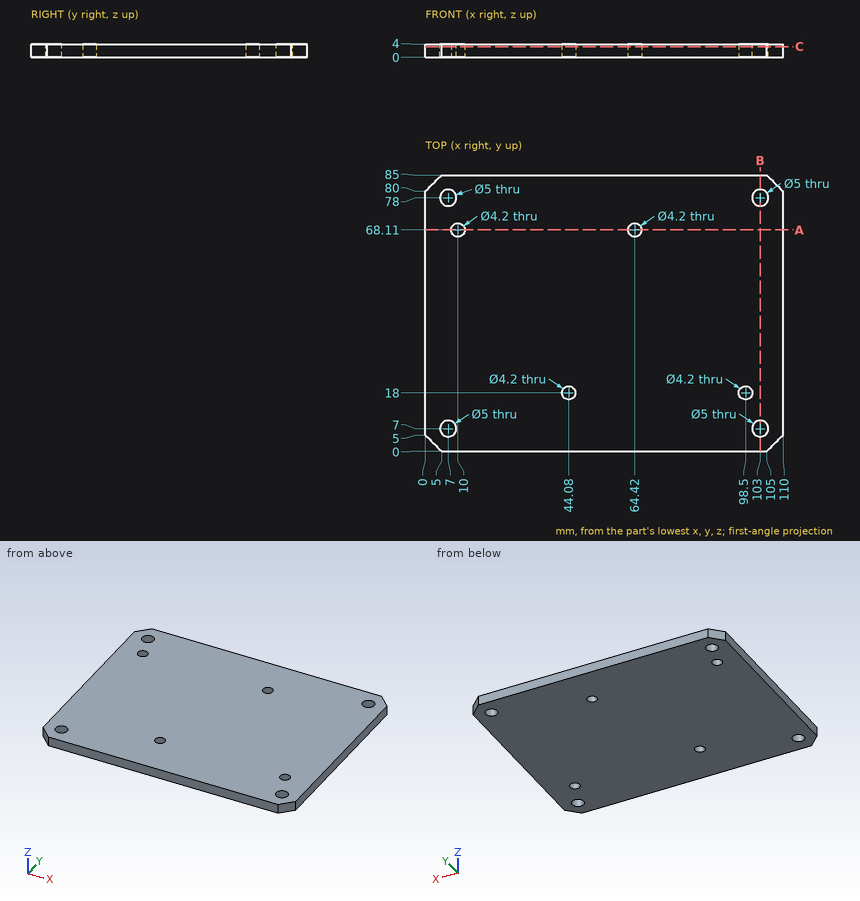
Could you check a few things on this drawing? It's one solid part, dimensions in mm from its lowest x, y, z. Give positions to 0.01 mm unless a question says otherwise; leave off trailing zeros. Write each loop counter-clockwise with the first axis right and the second up, starting at its lowest first coordinate (ties: lowest second). Pieces come first, ordered by that corner, then holes. Notation, with made-up numbers: (1.25, -29.5) - (27.25, -29.5) arc R22 cw to (27.25, -13.5) - close; hole circle Ø3 at (18.5, -28.5). An arc over 180 degrees is marked (long way). Use CSV: the item, a comma, the result in double quotes. Start each with the question number.
Item 1: If I drill on line 1 along Y through (x, z) = (7, 1.8); line 2 along Y through (x, z) = (98.5, 1.3); line 3 along Y through (x, z) = (64.42, 1.8), over which ranges is the centre line in solid material (lowest first)?
Item 2: I want a section at A-A, the plane y = 68.11. Please give me the cut outline in (x, z), then the cut area to 3 significant figures.
Item 3: I want a section at B-B, the plane x = 103. Please give me the cut outline in (y, z), then the cut area to 3 significant figures.
Item 4: I want a section at C-C, the plane z = 3.2. Give the number of separate pieces and of enclosed holes in the cut face, then the cut area to 3 significant figures.
Findings:
1,line 1,"y = 0 to 4.5, 9.5 to 75.5, 80.5 to 85"
1,line 2,"y = 0 to 15.9, 20.1 to 85"
1,line 3,"y = 0 to 66.01, 70.21 to 85"
2,outline,"(0, 0) - (7.9, 0) - (7.9, 4) - (0, 4) - close; (12.1, 0) - (62.32, 0) - (62.32, 4) - (12.1, 4) - close; (66.52, 0) - (110, 0) - (110, 4) - (66.52, 4) - close"
2,area,"406 mm2"
3,outline,"(0, 0) - (4.5, 0) - (4.5, 4) - (0, 4) - close; (9.5, 0) - (75.5, 0) - (75.5, 4) - (9.5, 4) - close; (80.5, 0) - (85, 0) - (85, 4) - (80.5, 4) - close"
3,area,"300 mm2"
4,separate pieces,"1"
4,enclosed holes,"8"
4,area,"9,170 mm2"
